from build123d import *

# Parameters (mm, degrees)
SKETCH1_W             = 54
SKETCH1_H             = 68
BOSS_EXTRUDE1_DEPTH   = 60
SKETCH2_W             = 106
SKETCH2_H             = 90
BOSS_EXTRUDE2_DEPTH   = 16
SKETCH3_W             = 78
SKETCH3_H             = 78
BOSS_EXTRUDE3_DEPTH   = 15
CHAMFER1_SIZE         = 5
SKETCH4_R             = 35.15
SKETCH4_R_2           = 31.35
CUT_EXTRUDE1_DEPTH    = 1.97
HOLE1_D               = 16
HOLE2_D               = 22
HOLE2_DEPTH           = 63
CHAMFER2_SIZE         = 1
M5_TAPPED_HOLE1_D     = 4.2
M5_TAPPED_HOLE1_DEPTH = 10
M5_TAPPED_HOLE1_TIP   = 1.2618073
HOLE3_D               = 6.4
HOLE3_CBORE_D         = 11
HOLE3_CBORE_DEPTH     = 9
SKETCH16_R            = 10.3
CUT_EXTRUDE2_DEPTH    = 3.8


with BuildPart() as part:
    # Sketch1 → Boss-Extrude1 (new body)
    with BuildSketch(Plane.XY):
        Rectangle(SKETCH1_W, SKETCH1_H)
    extrude(amount=BOSS_EXTRUDE1_DEPTH)

    # Sketch2 → Boss-Extrude2 (add)
    with BuildSketch(Plane.XY.offset(60)):
        Rectangle(SKETCH2_W, SKETCH2_H)
    extrude(amount=BOSS_EXTRUDE2_DEPTH)

    # Sketch3 → Boss-Extrude3 (add)
    with BuildSketch(Plane.XY.offset(76)):
        Rectangle(SKETCH3_W, SKETCH3_H)
    extrude(amount=BOSS_EXTRUDE3_DEPTH)

    # Chamfer1
    chamfer1_edges = [part.edges().sort_by_distance(p)[0] for p in [
        (-53, 45, 68),
        (-53, -45, 68),
        (53, -45, 68),
        (53, 45, 68),
        (-39, 39, 83.5),
        (-39, -39, 83.5),
        (39, -39, 83.5),
        (39, 39, 83.5),
        (27, -34, 30),
        (-27, -34, 30),
        (-27, 34, 30),
        (27, 34, 30),
    ]]
    chamfer(chamfer1_edges, length=CHAMFER1_SIZE)

    # Sketch4 → Cut-Extrude1 (cut)
    with BuildSketch(Plane.XY.offset(91)):
        Circle(SKETCH4_R)
        Circle(SKETCH4_R_2, mode=Mode.SUBTRACT)
    extrude(amount=-CUT_EXTRUDE1_DEPTH, mode=Mode.SUBTRACT)

    # Hole1 (through all)
    with Locations(Plane.XY.offset(91)):
        with Locations((0, -18), (0, 18)):
            Hole(HOLE1_D / 2)

    # Hole2
    with Locations(Plane(origin=(0, 0, 0), x_dir=(-1, 0, 0), z_dir=(0, 0, -1))):
        with Locations((0, 18), (0, -18)):
            Hole(HOLE2_D / 2, depth=HOLE2_DEPTH)

    # Chamfer2
    chamfer2_edges = [part.edges().sort_by_distance(p)[0] for p in [
        (8, 18, 91),
        (8, -18, 91),
        (-11, -18, 0),
        (-11, 18, 0),
    ]]
    chamfer(chamfer2_edges, length=CHAMFER2_SIZE)

    # M5 Tapped Hole1
    with Locations(Plane(origin=(0, 0, 0), x_dir=(-1, 0, 0), z_dir=(0, 0, -1))):
        with Locations((20, -18), (20, 18), (-20, 18), (-20, -18)):
            Hole(M5_TAPPED_HOLE1_D / 2, depth=M5_TAPPED_HOLE1_DEPTH)
            with Locations((0, 0, -(M5_TAPPED_HOLE1_DEPTH + M5_TAPPED_HOLE1_TIP / 2))):  # 118° drill point
                Cone(0, M5_TAPPED_HOLE1_D / 2, M5_TAPPED_HOLE1_TIP, mode=Mode.SUBTRACT)

    # Hole3 (through all)
    with Locations(Plane(origin=(0, 0, 60), x_dir=(-1, 0, 0), z_dir=(0, 0, -1))):
        with Locations((45, -30), (45, 30), (-45, 30), (-45, -30)):
            CounterBoreHole(HOLE3_D / 2, HOLE3_CBORE_D / 2, HOLE3_CBORE_DEPTH)

    # Sketch16 → Cut-Extrude2 (cut)
    with BuildSketch(Plane.XY.offset(86)):
        with Locations((0, 18)):
            Circle(SKETCH16_R)
        with Locations((0, -18)):
            Circle(SKETCH16_R)
    extrude(amount=-CUT_EXTRUDE2_DEPTH, mode=Mode.SUBTRACT)


solid = part.part
Check sheet for the modelled part. Datum: model origin and axes. Units: mm. A direction names the side the tool comes from. Give positions to 0.01 mm unless a question says otherwise; leave off trailing zeros. Order: outer loops, then holes, each group sorted by start corner. A loop starts at its lowest first (then second) coordinate and runs counter-clockwise, first axis right, second up. Notation, with made-up numbers: M 44.25,26 L 70.25,26 A32 cw 70.25,62 Z; hole C 41.25,-8.5 d1. An arc over 180 degrees is marked long. Answer as CSV lines item,"result". Start each with the question number.
Item 1: Gauge pin test, flat ends, axial feed: P1, Ø2, axis at x = 33.5, y = 9, coming from the -Z side; P2, Ø5.5, axis at x = 44.5, y = -30, coming from the -Z side; P3, Ø8.5, axis at x = -45, y = -30, coming from the +Z side. Record the tip position at first contact, or that the pin passes through.
Item 2: Cross-section at C-C on z = 48. Enter the section's corners in (x, y), plus the area to 3 significant figures.
Item 3: Cross-section at B-B on y = 0. Enter the section's corners in (x, z).
Item 4: Mould release check, pull along Z, two halves, no side actions. Record for faces 1 (the face through (-1, 45, 68)), 2 (the face through (-6.2, 12.7, 86)), 3 (the face through (-19.73, 18.25, 11.04)): +Z half, -Z half, draft (parallel to the pull), parting line (faces both ways), or undercut.
Item 5: Cross-section at A-A on x = 45. Enter the section's corners in (y, z), plus the area to 3 significant figures.
Item 6: Thickness scan on line 1 (Y direction, x = 45, z = 75.5); line 2 (Y direction, x = -45, z = 65); line 3 (X direction, y = -18.5, z = 30.5). Record the ranges inside material, lowest first. Write a range as [from, to].
Item 7: Cross-section at D-D on x = -30. Enter the section's corners in (y, z), plus the area to 3 significant figures.
Item 8: Tool access check on faces 4 (the face through (-2.38, 7.26, 32.43)), 5 (the face through (25, -31, 30)), 6 (the face through (-6.2, 12.7, 82.2)). Record the directions out of +Z, -Z, +X, -X, +Y, -Y that give a thin tool (end or side, any length) a straight path to the whole face; none if there is none.
Established:
1,P1,"stops at z = 60"
1,P2,"stops at z = 69"
1,P3,"stops at z = 76"
2,outline,"M -27,-29 L -22,-34 L 22,-34 L 27,-29 L 27,29 L 22,34 L -22,34 L -27,29 Z; hole C 0,-18 d22; hole C 0,18 d22"
2,area,"2,860 mm^2"
3,outline,"M -53,60 L -27,60 L -27,0 L 27,0 L 27,60 L 53,60 L 53,76 L 39,76 L 39,91 L 35.15,91 L 35.15,89.03 L 31.35,89.03 L 31.35,91 L -31.35,91 L -31.35,89.03 L -35.15,89.03 L -35.15,91 L -39,91 L -39,76 L -53,76 Z"
4,face 1,"draft"
4,face 2,"undercut"
4,face 3,"-Z half"
5,outline,"M -45,60 L -35.5,60 L -35.5,69 L -33.2,69 L -33.2,76 L -45,76 Z; M -26.8,69 L -24.5,69 L -24.5,60 L 24.5,60 L 24.5,69 L 26.8,69 L 26.8,76 L -26.8,76 Z; M 33.2,69 L 35.5,69 L 35.5,60 L 45,60 L 45,76 L 33.2,76 Z"
5,area,"1,150 mm^2"
6,line 1,"y = [-45, -33.2], [-26.8, 26.8], [33.2, 45]"
6,line 2,"y = [-45, -35.5], [-24.5, 24.5], [35.5, 45]"
6,line 3,"x = [-27, -10.99], [10.99, 27]"
7,outline,"M -45,60 L 45,60 L 45,76 L 39,76 L 39,91 L 18.32,91 L 18.32,89.03 L 9.1,89.03 L 9.1,91 L -9.1,91 L -9.1,89.03 L -18.32,89.03 L -18.32,91 L -39,91 L -39,76 L -45,76 Z"
7,area,"2,570 mm^2"
8,face 4,"-Z"
8,face 5,"-Z, +X, -Y"
8,face 6,"none"
